For this review, use the dimensioned drawing (mm, ordinates from the lowest corner) and the shaded views. Coordinates: 2 decimals unless noted, no trailing zeros. Write each loop counter-clockwise with the first axis right and the second up, starting at its lowest first coordinate (ties: lowest second). Pieces come first, ordered by that corner, then holes. Notation, with made-up numbers: (40.25, -9.75) -> (79.25, -9.75) arc R17 ccw to (79.25, 12.25) -> close; hole circle Ø10 at (47, -10.5). An arc over 180 degrees is marked (long way). Put each result on its own line as item: value. Start each with the question number.
Item 1: To check wall thickness, follow L1, parallel to Y at x = 8, z = 0.5 (1 decimal); L2, parallel to Y at x = 6.5, z = 3 (1 decimal); L3, parallel to X at y = 3, z = 4.5 (1 decimal). State the ranges of each line that lie inside material, in increasing order.
Item 2: Consider section A-A on z = 4. Give the boundary of the cut face in (x, y).
Item 3: Consider section B-B on z = 0.75. Give the boundary of the cut face in (x, y).
Item 4: Insertion check: P1, Ø1.5, axis at x = 9, z = 3, coming from the +Y side. The pin has a flat end and moves straight along its axis. Give the tip position at first contact, or say it passes through.
Item 5: The part is to be moulded in two halves that separate along Y. For the marked faces 1, 2, 3 and 4, say which applies: +Y half, -Y half, draft (parallel to the pull), parting line (faces both ways), or undercut.
Item 6: Consider section C-C on z = 6. Give the boundary of the cut face in (x, y) (1 decimal).
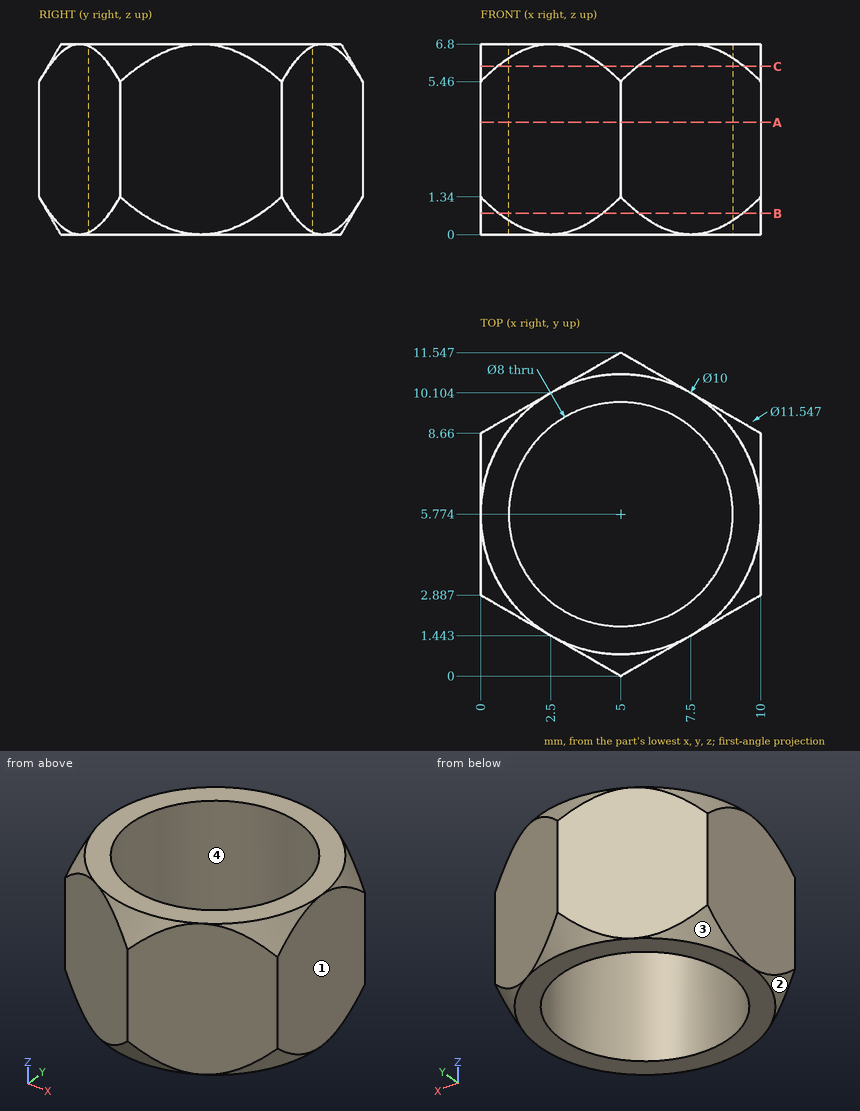
Return value:
1. L1: 1.7 to 3.1, 8.4 to 9.8
1. L2: 0.9 to 2.1, 9.5 to 10.7
1. L3: 0 to 2.1, 7.9 to 10
2. outline: (0, 2.89) -> (5, 0) -> (10, 2.89) -> (10, 8.66) -> (5, 11.55) -> (0, 8.66) -> close; hole circle Ø8 at (5, 5.77)
3. outline: (0, 3.65) arc R5.43 ccw to (0.66, 2.51) -> (4.34, 0.38) arc R5.43 ccw to (5.66, 0.38) -> (9.34, 2.51) arc R5.43 ccw to (10, 3.65) -> (10, 7.9) arc R5.43 ccw to (9.34, 9.04) -> (5.66, 11.17) arc R5.43 ccw to (4.34, 11.17) -> (0.66, 9.04) arc R5.43 ccw to (0, 7.9) -> close; hole circle Ø8 at (5, 5.77)
4. P1: y = 9.67
5. face 1: draft
5. face 2: -Y half
5. face 3: +Y half
5. face 4: undercut
6. outline: (0, 3.6) arc R5.5 ccw to (0.6, 2.5) -> (4.4, 0.3) arc R5.5 ccw to (5.6, 0.3) -> (9.4, 2.5) arc R5.5 ccw to (10, 3.6) -> (10, 8) arc R5.5 ccw to (9.4, 9) -> (5.6, 11.2) arc R5.5 ccw to (4.4, 11.2) -> (0.6, 9) arc R5.5 ccw to (0, 8) -> close; hole circle Ø8 at (5, 5.8)
